Work out the finished part from the listing and answer in its coordinate system (mm). Face numbers are marked on the shaded views. A direction names the side the tool comes from. Coordinates: 2 decimals unless noted, no trailing zeros. Order: outer loops, then holes, each group sorted by start corner. A loop starts at its lowest first (then second) coordinate and runs counter-clockwise, first axis right, second up. Notation, with made-up numbers: (21, -13) - (45, -13) arc R25 ccw to (45, -1) - close; hole circle Ø1 at (82.25, 70.25). An arc over 180 degrees is marked (long way). Answer as a JSON object with one key per item and string values. Group by question number.
1) Find the intervals of material crossed by line 1 along X through (y, z) = (-8, -16.5); line 2 along Y through (x, z) = (0.75, 0); line 3 along Y through (x, z) = (-7, 0), in increasing order.
2) Section A-A (x = -1.25) is taken. Give the vertices of the cut face in (y, z).
3) The mould has two halves that part along Z. Classify the marked faces 4, 5 and 6: released by +Z, released by -Z, zero draft, split by the parting line, or undercut.
4) A tool of negligible diameter and unlimited length cuts with its end or side. For the marked faces 1, 2 and 3, from which of +Z, -Z, +X, -X, +Y, -Y can it reach the whole face along a straight path? Write none if from no direction.
5) Each of these flat-tipped pins is pushed along its axis until it touches: P1, Ø13, axis at y = -0.5, z = 0.5, coming from the -X side; P2, Ø1.5, axis at x = 2, y = 6.5, coming from the +Z side; P3, Ø12, axis at x = -9, y = -8, coming from the +Z side; P4, Ø10, axis at x = 9.5, z = 17, coming from the +Y side. Where does it stop, or does it pass through?
from build123d import *

# Parameters (mm, degrees)
CHAMFER_1_SIZE = 0.5
FILLET_1_R     = 0.2


with BuildPart() as part:
    # 草图1 → 旋转1 (revolve)
    with BuildSketch(Plane.XY, mode=Mode.PRIVATE) as revolve_1_sk:
        Polygon((-13, 13), (-13, 23), (-10, 23), (-10, 18), (10, 18), (10, 23), (13, 23), (13, 13), (5, 13), (5, 10.5), (-5, 10.5), (-5, 13), align=None)
    revolve(revolve_1_sk.sketch.rotate(Axis((0, 0, 0), (1, 0, 0)), 90), axis=Axis((0, 0, 0), (1, 0, 0)))

    # 倒角1
    chamfer_1_edges = [part.edges().sort_by_distance(p)[0] for p in [
        (13, 0, -13),
        (13, 0, -23),
        (10, 0, -23),
        (-10, 0, -23),
        (-13, 0, -23),
        (-13, 0, -13),
        (-5, 0, -10.5),
        (5, 0, -10.5),
    ]]
    chamfer(chamfer_1_edges, length=CHAMFER_1_SIZE)

    # 圆角1
    fillet_1_edges = [part.edges().sort_by_distance(p)[0] for p in [
        (10, 0, -18),
        (-10, 0, -18),
        (-5, 0, -13),
        (5, 0, -13),
    ]]
    fillet(fillet_1_edges, radius=FILLET_1_R)


solid = part.part
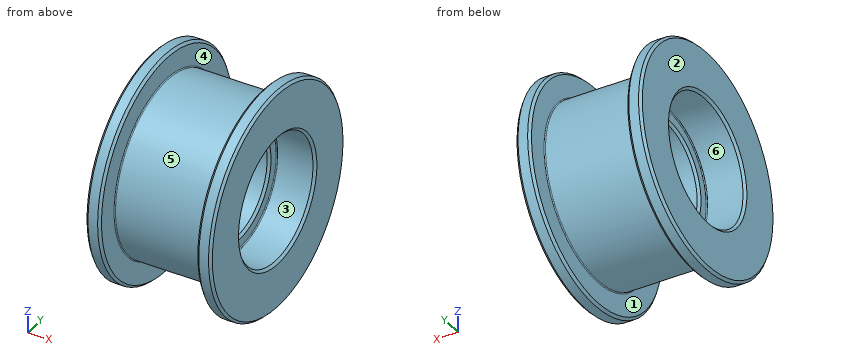
Report:
{
 "1": {"line 1": "x = -13 to -10, 10 to 13", "line 2": "y = -18 to -10.5, 10.5 to 18", "line 3": "y = -18 to -13, 13 to 18"},
 "2": {"outline": "circle Ø36 at (0, 0); hole circle Ø21 at (0, 0)"},
 "3": {"face 4": "zero draft", "face 5": "split by the parting line", "face 6": "undercut"},
 "4": {"face 1": "none", "face 2": "+Z, -Z, -X, +Y, -Y", "face 3": "+X"},
 "5": {"P1": "passes through", "P2": "stops at z = 17.06", "P3": "stops at z = 22.9", "P4": "stops at y = 19.56"}
}
